Design review of the part built by this model. Coordinates are the model's own, in mm. A direction names the side the tool comes from. Round coordinates to 2 decimals unless told otherwise and drop trailing zeros. Write each loop counter-clockwise with the first axis right and the second up, starting at its lowest first coordinate (ties: lowest second). Pieces come first, ordered by that corner, then holes. Notation, with made-up numbers: (5.25, -30.75) -> (57.25, -30.75) arc R25 cw to (57.25, -16.75) -> close; hole circle Ø1 at (-24, 41.25). An arc over 180 degrees is marked (long way). One line per question, with ' | ' between items. Start each with the question number.
1) For faces 4 (the cylindrical face through (32.17, -52.55, -6.9)), 5 (the cylindrical face through (14.93, 38.88, -39.74)), 6 (the flat face through (40.6, -15, -45)), list the 3-axis set-ups (+Z, -Z, +X, -X, +Y, -Y) from which the entire face can be reached by the end or side of a thin tool; tool diameter is ignored.
2) Mouldability with a two-part tool opening along Z and no side actions: class faces 1 (the flat face through (20, 53, 10)), 2 (the cylindrical face through (15.07, -19.52, 62)), 3 (the cylindrical face through (14.93, -0.766, -55.653)) as +Z half, -Z half, draft (parallel to the pull), parting line (faces both ways), or undercut.
3) For probe 1 along X at (y, z) = (48.5, 5.5); probe 2 along X at (y, z) = (-13.5, -44); probe 3 along Y at (x, z) = (41, 0), list the stretches that pass through material, from the lowest coordinate up.
4) Consider section C-C (x = 18.5). Count the separate pieces of the cut face and the enclosed holes in it, then the cut area to 3 significant figures.
5) Insertion check: pin 1 Ø10 at (x, z) = (39, -20) entering from +Y; pin 2 Ø12 at (x, y) = (19.5, -23) entering from -Z; pin 3 Ø5 at (y, z) = (40.66, 40.66) entering from -X; pin 4 Ø2.5 at (y, z) = (-57.5, 0) entering from -X. Each pin has a flat end and moves straight along its axis. Give the tip position at first contact, or say it passes through.
6) Consider section D-D (x = 34.5). Give the boundary of the cut face in (y, z), then the cut area to 3 significant figures.
7) Consider section A-A (z = 57.5). Give the boundary of the cut face in (x, y), then the cut area to 3 significant figures.
```python
from build123d import *

# Parameters (mm, degrees)
SKETCH_2_W          = 20
SKETCH_2_H          = 65
SKETCH_3_W          = 25
SKETCH_3_H          = 53
SKETCH_6_R          = 35
CUT_EXTRUDE_1_DEPTH = 103.347447452
CUT_EXTRUDE_START   = 13.2
SKETCH_7_R          = 47
CUT_EXTRUDE_2_DEPTH = 90.147447452
CUT_EXTRUDE_START_2 = 40.6
SKETCH_10_R         = 50.5
CUT_EXTRUDE_4_DEPTH = 3.4
SKETCH_15_R         = 65
CUT_EXTRUDE_6_DEPTH = 10
CUT_EXTRUDE_START_3 = 44.6
SKETCH_12_R         = 49.5
CUT_EXTRUDE_5_DEPTH = 58.747447452
SKETCH_16_R         = 2
CUT_EXTRUDE_7_DEPTH = 99.361577865
CHAMFER_1_SIZE      = 1


with BuildPart() as part:
    # 草图2 → 旋转-薄壁1 (revolve)
    with BuildSketch(Plane.XY, mode=Mode.PRIVATE) as revolve_1_sk:
        with Locations((10, 32.5)):
            Rectangle(SKETCH_2_W, SKETCH_2_H)
    revolve(revolve_1_sk.sketch.rotate(Axis((0, 0, 0), (1, 0, 0)), 90), axis=Axis((0, 0, 0), (1, 0, 0)))

    # 草图3 → 旋转-薄壁2 (revolve)
    with BuildSketch(Plane.XY, mode=Mode.PRIVATE) as revolve_2_sk:
        with Locations((32.5, 26.5)):
            Rectangle(SKETCH_3_W, SKETCH_3_H)
    revolve(revolve_2_sk.sketch.rotate(Axis((20, 0, 0), (1, 0, 0)), 90), axis=Axis((20, 0, 0), (1, 0, 0)))

    # 草图6 → 切除-拉伸1 (cut, through all)
    with BuildSketch(Plane(origin=(0, 0, 0), x_dir=(0, 0, -1), z_dir=(1, 0, 0))):
        with Locations(Location((0, 0, 0), (0, 0, 180))):
            Circle(SKETCH_6_R)
    extrude(amount=CUT_EXTRUDE_1_DEPTH, mode=Mode.SUBTRACT)

    # 草图7 → 切除-拉伸2 (cut, through all)
    with BuildSketch(Plane(origin=(0, 0, 0), x_dir=(0, 0, -1), z_dir=(1, 0, 0)).offset(CUT_EXTRUDE_START)):
        Circle(SKETCH_7_R)
    extrude(amount=CUT_EXTRUDE_2_DEPTH, mode=Mode.SUBTRACT)

    # 草图10 → 切除-拉伸4 (cut)
    with BuildSketch(Plane(origin=(0, 0, 0), x_dir=(0, 0, -1), z_dir=(1, 0, 0)).offset(CUT_EXTRUDE_START_2)):
        Circle(SKETCH_10_R)
    extrude(amount=-CUT_EXTRUDE_4_DEPTH, mode=Mode.SUBTRACT)

    # 草图15 → 切除-拉伸6 (cut)
    with BuildSketch(Plane(origin=(0, 0, 0), x_dir=(0, 0, -1), z_dir=(1, 0, 0))):
        with Locations(Location((0, 0, 0), (0, 0, 180))):
            Circle(SKETCH_15_R)
    extrude(amount=CUT_EXTRUDE_6_DEPTH, mode=Mode.SUBTRACT)

    # 草图12 → 切除-拉伸5 (cut, through all)
    with BuildSketch(Plane(origin=(0, 0, 0), x_dir=(0, 0, -1), z_dir=(1, 0, 0)).offset(CUT_EXTRUDE_START_3)):
        Circle(SKETCH_12_R)
    extrude(amount=CUT_EXTRUDE_5_DEPTH, mode=Mode.SUBTRACT)

    # 草图16 → 切除-拉伸7 (cut, through all)
    with BuildSketch(Plane.ZY.offset(-10)):
        with Locations((0, 57.5)):
            Circle(SKETCH_16_R)
        with Locations((40.658639918, 40.658639918)):
            Circle(SKETCH_16_R)
        with Locations((57.5, 0)):
            Circle(SKETCH_16_R)
        with Locations((40.658639918, -40.658639918)):
            Circle(SKETCH_16_R)
        with Locations((0, -57.5)):
            Circle(SKETCH_16_R)
        with Locations((-40.658639918, -40.658639918)):
            Circle(SKETCH_16_R)
        with Locations((-57.5, 0)):
            Circle(SKETCH_16_R)
        with Locations((-40.658639918, 40.658639918)):
            Circle(SKETCH_16_R)
    extrude(amount=-CUT_EXTRUDE_7_DEPTH, mode=Mode.SUBTRACT)

    # 倒角1
    chamfer_1_edges = [part.edges().sort_by_distance(p)[0] for p in [
        (45, 0, -53),
    ]]
    chamfer(chamfer_1_edges, length=CHAMFER_1_SIZE)


solid = part.part
```
From the geometry:
1) face 4: +X | face 5: +X, -X | face 6: none
2) face 1: draft | face 2: parting line | face 3: undercut
3) probe 1: x = 10 to 37.2, 40.6 to 44.6 | probe 2: x = 10 to 13.2 | probe 3: y = -53 to -47, 47 to 53
4) separate pieces: 1 | enclosed holes: 9 | area: 6,230 mm2
5) pin 1: stops at y = 50.83 | pin 2: stops at z = -62.74 | pin 3: stops at x = 10 | pin 4: passes through
6) outline: circle Ø106 at (0, 0); hole circle Ø94 at (0, 0) | area: 1,880 mm2
7) outline: (10, -30.31) -> (20, -30.31) -> (20, -2) -> (10, -2) -> close; (10, 2) -> (20, 2) -> (20, 30.31) -> (10, 30.31) -> close | area: 566 mm2
